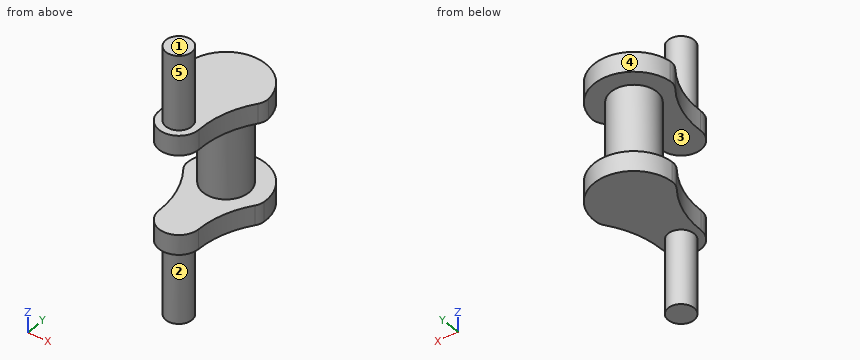
from build123d import *

# Parameters (mm, degrees)
FRONT_PLATE_DEPTH      = 20
FRONT_PIN_PROFILE_26_R = 13
FRONT_PIN_26_DEPTH     = 75
JOURNAL_PROFILE_46_R   = 23
JOURNAL_46_DEPTH       = 80
REAR_START             = -20
REAR_PLATE_DEPTH       = 20
REAR_START_2           = 75
REAR_PIN_PROFILE_26_R  = 13
REAR_PIN_26_DEPTH      = 75


with BuildPart() as part:
    # Front Plate Profile → Front Plate (new body)
    with BuildSketch(Plane.XY):
        with BuildLine():
            ThreePointArc((-19.989200766, 0.657155043), (-0.067809086, -19.999885048), (19.993197289, 0.52159577))
            ThreePointArc((19.993197289, 0.52159577), (23.983612751, 29.469835271), (37.03816485, 55.613718978))
            ThreePointArc((37.03816485, 55.613718978), (39.360775458, 60.47698398), (39.814551695, 65.847268297))
            ThreePointArc((39.814551695, 65.847268297), (0.541840926, 101.996329937), (-39.695719365, 66.9244151))
            ThreePointArc((-39.695719365, 66.9244151), (-39.339964644, 61.352839249), (-36.971364547, 56.297272766))
            ThreePointArc((-36.971364547, 56.297272766), (-23.860759515, 29.887158775), (-19.989200766, 0.657155043))
        make_face()
    extrude(amount=FRONT_PLATE_DEPTH)

    # Front Pin Profile Ø26 → Front Pin Ø26 (add)
    with BuildSketch(Plane.XY.offset(20)):
        Circle(FRONT_PIN_PROFILE_26_R)
    extrude(amount=FRONT_PIN_26_DEPTH)

    # Journal Profile Ø46 → Journal Ø46 (add)
    with BuildSketch(Plane(origin=(0, 0, 0), x_dir=(-1, 0, 0), z_dir=(0, 0, -1))):
        with Locations(Location((0, 62, 0), (0, 0, 180))):
            Circle(JOURNAL_PROFILE_46_R)
    extrude(amount=JOURNAL_46_DEPTH)

    # Rear Plate Profile → Rear Plate (add)
    with BuildSketch(Plane.XY.offset(-80).offset(REAR_START)):
        with BuildLine():
            ThreePointArc((-19.997507027, 0.315773186), (-0.260135851, -19.998308162), (19.998954502, -0.204496502))
            ThreePointArc((19.998954502, -0.204496502), (24.520770215, 27.058319007), (37.101446898, 51.663897663))
            ThreePointArc((37.101446898, 51.663897663), (39.072985568, 55.400775042), (39.924234273, 59.539203839))
            ThreePointArc((39.924234273, 59.539203839), (2.310034684, 101.933241038), (-39.941678501, 64.159240274))
            ThreePointArc((-39.941678501, 64.159240274), (-39.351963031, 59.110003561), (-37.109654718, 54.547700507))
            ThreePointArc((-37.109654718, 54.547700507), (-24.157614064, 28.818824435), (-19.997507027, 0.315773186))
        make_face()
    extrude(amount=REAR_PLATE_DEPTH)

    # Rear Pin Profile Ø26 → Rear Pin Ø26 (add)
    with BuildSketch(Plane(origin=(0, 0, -100), x_dir=(-1, 0, 0), z_dir=(0, 0, -1)).offset(REAR_START_2)):
        with Locations(Location((0, 0, 0), (0, 0, 180))):
            Circle(REAR_PIN_PROFILE_26_R)
    extrude(amount=-REAR_PIN_26_DEPTH)


solid = part.part
Design review of the part built by this model. Coordinates are the model's own, in mm. Face numbers are marked on the shaded views. A direction names the side the tool comes from. Round coordinates to 2 decimals unless told otherwise and drop trailing zeros. Loops run counter-clockwise (first coordinate to the right, second up) from the corner with the lowest first, then second, coordinate; pieces in that order, holes last. Notation, with made-up numbers: (-11.75, 36.5) -> (29.25, 36.5) arc R15 cw to (29.25, 57.5) -> close; hole circle Ø10 at (47.5, -23.5). An arc over 180 degrees is marked (long way). Use one line per item in the form item = value. Start each with the question number.
Q1. We need section D-D on y = 44.5. Give the boundary of the cut face in (x, z), then the cut area to 3 significant figures.
Q2. We need section B-B on x = 0. Give the boundary of the cut face in (y, z), then the cut area to 3 significant figures.
Q3. We need section A-A on y = 32. Give the boundary of the cut face in (x, z).
Q4. For pin 1 Ø10 at (x, y) = (-16, 84.5) entering from +Z; pin 2 Ø2 at (y, z) = (8, 24) entering from -X; pin 3 Ø6 at (y, z) = (-4, 48.5) entering from +X, all flat-tipped, find the tip position at first contact; note any pin that passes through.
Q5. Wall thickness on line 1 along Z through (x, y) = (17.5, 97); line 2 along Z through (x, y) = (3, -2.5); line 3 along X through (y, z) = (6, 19): over which ranges is each line inside the solid? List them lowest first. Write a range as [from, to].
Q6. Machinability: for the marked faces 1, 2, 3, 4 and 5, which of the approach directions +Z, -Z, +X, -X, +Y, -Y give a long, thin tool a straight path to every point of the face, cutting with its end or side? Answer none if there is none.
Calculated:
q1.outline = (-30.79, -100) -> (32.42, -100) -> (32.42, -80) -> (14.92, -80) -> (14.92, 0) -> (30.17, 0) -> (30.17, 20) -> (-29.76, 20) -> (-29.76, 0) -> (-14.92, 0) -> (-14.92, -80) -> (-30.79, -80) -> close
q1.area = 4,850 mm²
q2.outline = (-20, -100) -> (-13, -100) -> (-13, -175) -> (13, -175) -> (13, -100) -> (102, -100) -> (102, -80) -> (85, -80) -> (85, 0) -> (102, 0) -> (102, 20) -> (13, 20) -> (13, 95) -> (-13, 95) -> (-13, 20) -> (-20, 20) -> (-20, 0) -> (39, 0) -> (39, -80) -> (-20, -80) -> close
q2.area = 12,500 mm²
q3.outline = (-25.23, -100) -> (26.31, -100) -> (26.31, -80) -> (-25.23, -80) -> close; (-24.53, 0) -> (24.81, 0) -> (24.81, 20) -> (-24.53, 20) -> close
q4.pin_1 = 20
q4.pin_2 = -10.95
q4.pin_3 = 12.96
q5.line_1 = [-100, -80], [0, 20]
q5.line_2 = [-175, -80], [0, 95]
q5.line_3 = [-19.97, 20.02]
q6.face_1 = +Z, +X, -X, +Y, -Y
q6.face_2 = -Z
q6.face_3 = none
q6.face_4 = +Z, -Z, +Y
q6.face_5 = +Z
